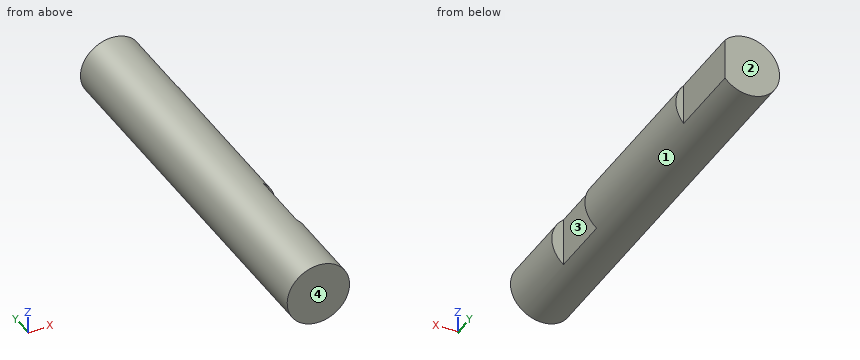
from build123d import *

# Parameters (mm, degrees)
SKETCH1_R               = 8
BOSS_EXTRUDE1_DEPTH     = 100
CUT_EXTRUDE1_DEPTH      = 101.637965003
CUT_EXTRUDE1_DEPTH_BACK = 101.637965003
SKETCH2_W               = 2
SKETCH2_H               = 20
SKETCH2_W_2             = 6
SKETCH2_H_2             = 16


with BuildPart() as part:
    # Sketch1 → Boss-Extrude1 (new body)
    with BuildSketch(Plane(origin=(0, 0, 0), x_dir=(1, 0, 0), z_dir=(0, 1, 0))):
        with Locations(Location((0, 0, 0), (0, 0, 270))):
            Circle(SKETCH1_R)
    extrude(amount=BOSS_EXTRUDE1_DEPTH)

    # Sketch2 → Cut-Extrude1 (cut, two sides: drawn at the far end of the back side and taken through both)
    with BuildSketch(Plane.XY.offset(-CUT_EXTRUDE1_DEPTH_BACK)):
        with Locations((7, 90)):
            Rectangle(SKETCH2_W, SKETCH2_H)
        with Locations((8, 28)):
            Rectangle(SKETCH2_W_2, SKETCH2_H_2)
    extrude(amount=CUT_EXTRUDE1_DEPTH + CUT_EXTRUDE1_DEPTH_BACK, mode=Mode.SUBTRACT)


solid = part.part
Design review of the part built by this model. Coordinates are the model's own, in mm. Face numbers are marked on the shaded views. Coordinates: 2 decimals unless noted, no trailing zeros. Loops run counter-clockwise (first coordinate to the right, second up) from the corner with the lowest first, then second, coordinate; pieces in that order, holes last.
Item 1: Add section B-B (y = 82.5). Write out the cut boundary in (x, z), and give its area (3 significant figures).
Completed:
outline: (6, -5.29) - (6, 5.29) arc R8 ccw (long way) to start
area: 187 mm2
Item 2: Wall thickness on L1, parallel to Z at x = 0.5, y = 8.5; L2, parallel to X at y = 23, z = -0.5: over which ranges is each line inside the solid? List them lowest first.
Completed:
L1: z = -7.98 to 7.98
L2: x = -7.98 to 5
Item 3: Clearance check with flat-ended pins moving along their axes: pin 1 (3 mm diameter, centred on y = 89, z = 1, fed in from +X); pin 2 (3.5 mm diameter, centred on y = 28, z = -2, fed in from +X); pin 3 (3 mm diameter, centred on y = 76.5, z = -5, fed in from -X). State where each tip first meets the part, or that it passes through.
Completed:
pin 1: stops at x = 6
pin 2: stops at x = 5
pin 3: stops at x = -7.19
Item 4: Add section D-D (z = 3.75). Write out the cut boundary in (x, y).
Completed:
outline: (-7.07, 0) - (7.07, 0) - (7.07, 20) - (5, 20) - (5, 36) - (7.07, 36) - (7.07, 80) - (6, 80) - (6, 100) - (-7.07, 100) - close
Item 5: Add section C-C (x = -6.5). Write out the cut boundary in (y, z), and give its area (3 significant figures).
Completed:
outline: (0, -4.66) - (100, -4.66) - (100, 4.66) - (0, 4.66) - close
area: 933 mm2
Item 6: Add section A-A (z = 0). Write out the cut boundary in (x, y), and give its area (3 significant figures).
Completed:
outline: (-8, 0) - (8, 0) - (8, 20) - (5, 20) - (5, 36) - (8, 36) - (8, 80) - (6, 80) - (6, 100) - (-8, 100) - close
area: 1,510 mm2
Item 7: Draft analysis for pull direction Y (two halves, no side actions). For the marked faces 1, 2, 3 and 4, state which applies: pulls with the +Y half, pulls with the -Y half, needs draft (parallel to the pull), parting line crosses it, or undercut.
Completed:
face 1: needs draft
face 2: pulls with the +Y half
face 3: undercut
face 4: pulls with the -Y half
